Build history of the part. All positions in model axes, mm. Give positions to 0.01 mm unless a question says otherwise; leave off trailing zeros. Loops run counter-clockwise (first coordinate to the right, second up) from the corner with the lowest first, then second, coordinate; pieces in that order, holes last. Notation, with made-up numbers: (-21, 19.5) - (-16, 19.5) arc R22 ccw to (-16, 27.5) - close; hole circle Ø9 at (-28, -1). An arc over 180 degrees is marked (long way). Return JSON: item names as keys, results as strings. Group by question number.
1) Mould opens along X. For faces 1 (the face through (7, 0, 50)), 2 (the face through (31, 9.76, 24.66)), 3 (the face through (-1.19, -5.37, 24.66)) say: released by +X, released by -X, zero draft, split by the parting line, or undercut.
2) Drop flat-ended pins along their axis: pin 1 (12 mm diameter, centred on y = -13, z = 27.5, fed in from +X); pin 2 (10 mm diameter, centred on y = -24.5, z = 40.5, fed in from -X); pin 3 (1 mm diameter, centred on y = 9, z = 18.5, fed in from +X). Give the stop position or say it passes through.
3) Slice it at A-A (x = 0). List the corners of the cut face in (y, z), and give its area (3 significant figures).
4) Slice it at C-C (z = 6.5). List the corners of the cut face in (x, y).
5) Drill centre lines: probe 1 along Y at (x, z) = (0, 38); probe 2 along Y at (x, z) = (6, 41.5); probe 3 along Y at (x, z) = (28.5, 12). Where is each one in solid material? Low to high. Write a range as from..to.
```python
from build123d import *

# Parameters (mm, degrees)
SKETCH_1_R      = 32.5
SKETCH_1_R_2    = 5.5
EXTRUDE_1_DEPTH = 50
CHAMFER_1_SIZE  = 1


with BuildPart() as part:
    # 草图1 → 凸台-拉伸1 (new body)
    with BuildSketch(Plane.XY):
        Circle(SKETCH_1_R)
        Circle(SKETCH_1_R_2, mode=Mode.SUBTRACT)
    extrude(amount=EXTRUDE_1_DEPTH)

    # 倒角1
    chamfer_1_edges = [part.edges().sort_by_distance(p)[0] for p in [
        (-32.5, 0, 0),
        (-32.5, 0, 50),
        (-5.5, 0, 0),
        (-5.5, 0, 50),
    ]]
    chamfer(chamfer_1_edges, length=CHAMFER_1_SIZE)


solid = part.part
```
Results:
{
 "1": {"face 1": "zero draft", "face 2": "split by the parting line", "face 3": "undercut"},
 "2": {"pin 1": "x = 31.74", "pin 2": "x = -26", "pin 3": "x = 31.37"},
 "3": {"outline": "(-32.5, 1) - (-31.5, 0) - (-6.5, 0) - (-5.5, 1) - (-5.5, 49) - (-6.5, 50) - (-31.5, 50) - (-32.5, 49) - close; (5.5, 1) - (6.5, 0) - (31.5, 0) - (32.5, 1) - (32.5, 49) - (31.5, 50) - (6.5, 50) - (5.5, 49) - close", "area": "2,700 mm2"},
 "4": {"outline": "circle Ø65 at (0, 0); hole circle Ø11 at (0, 0)"},
 "5": {"probe 1": "-32.5..-5.5, 5.5..32.5", "probe 2": "-31.94..31.94", "probe 3": "-15.62..15.62"}
}
